Part model, mm, in its own coordinate system. A direction names the side the tool comes from. Coordinates: 2 decimals unless noted, no trailing zeros. Loops run counter-clockwise (first coordinate to the right, second up) from the corner with the lowest first, then second, coordinate; pieces in that order, holes last. Notation, with made-up numbers: (40, 29) -> (96, 29) arc R28 ccw to (96, 50) -> close; hole circle Ø8 at (40, 27). An arc over 180 degrees is marked (long way). One line per item, written item: value. Start each with the question number.
from build123d import *

# Parameters (mm, degrees)
SKETCH_1_R             = 3
EXTRUDE_1_DEPTH        = 71
HOLE_WIZARD_M4_2_D     = 3.3
HOLE_WIZARD_M4_2_DEPTH = 11.5
HOLE_WIZARD_M4_2_TIP   = 0.991420021
CHAMFER_1_SIZE         = 0.5
EXTRUDE1_DEPTH         = 72.126647608
EXTRUDE1_DEPTH_BACK    = 72.126647608
SKETCH1_W              = 2.697137816
SKETCH1_H              = 6
SKETCH1_W_2            = 2.361838602
SKETCH4_R              = 5
SKETCH4_R_2            = 3
EXTRUDE2_DEPTH         = 3


with BuildPart() as part:
    # 草图1 → 凸台-拉伸1 (new body)
    with BuildSketch(Plane.XY):
        Circle(SKETCH_1_R)
    extrude(amount=EXTRUDE_1_DEPTH)

    # M4 螺纹孔2
    with Locations(Plane.XY.offset(71)):
        with Locations((0, 0)):
            Hole(HOLE_WIZARD_M4_2_D / 2, depth=HOLE_WIZARD_M4_2_DEPTH)
            with Locations((0, 0, -(HOLE_WIZARD_M4_2_DEPTH + HOLE_WIZARD_M4_2_TIP / 2))):  # 118° drill point
                Cone(0, HOLE_WIZARD_M4_2_D / 2, HOLE_WIZARD_M4_2_TIP, mode=Mode.SUBTRACT)

    # 倒角1
    chamfer_1_edges = [part.edges().sort_by_distance(p)[0] for p in [
        (-3, 0, 71),
    ]]
    chamfer(chamfer_1_edges, length=CHAMFER_1_SIZE)

    # Sketch1 → Extrude1 (cut, two sides: drawn at the far end of the back side and taken through both)
    with BuildSketch(Plane(origin=(0, 0, 0), x_dir=(1, 0, 0), z_dir=(0, 1, 0)).offset(-EXTRUDE1_DEPTH_BACK)):
        with Locations((-3.848568908, -63)):
            Rectangle(SKETCH1_W, SKETCH1_H)
        with Locations((3.680919301, -63)):
            Rectangle(SKETCH1_W_2, SKETCH1_H)
    extrude(amount=EXTRUDE1_DEPTH + EXTRUDE1_DEPTH_BACK, mode=Mode.SUBTRACT)

    # Sketch4 → Extrude2 (add)
    with BuildSketch(Plane(origin=(0, 0, 0), x_dir=(-1, 0, 0), z_dir=(0, 0, -1))):
        Circle(SKETCH4_R)
        Circle(SKETCH4_R_2, mode=Mode.SUBTRACT)
    extrude(amount=-EXTRUDE2_DEPTH)


solid = part.part
1) Slice it at A-A (x = -4.25). Give the cut face in (y, z).
2) Pin check, flat tips, straight feed: pin 1 Ø3.5 at (y, z) = (-0.5, 62) entering from +X; pin 2 Ø1 at (x, z) = (2.5, 41) entering from +Y; pin 3 Ø3 at (y, z) = (1.5, 13.5) entering from +X. Stop position of each tip, or through.
3) Probe line 1 (Y direction, x = 0, z = 68.5); line 2 (X direction, y = 0, z = 63.75); line 3 (Z direction, x = -2, y = -4). List the from-to ranges inside material, lowest first. Write a range as from..to.
4) Tool access for faces 5 (the cylindrical face through (-3, 0, 36)), 6 (the flat face through (-2.5, 0, 63)), 7 (the flat face through (2, -1, 71)): list every direction of +Z, -Z, +X, -X, +Y, -Y with a clear straight run to the whole face (end or side of a thin tool).
5) Pull direction Y, two halves, no side cores. Call faces 1 (the conical face through (-0.1, -0.3, 58.7)), 2 (the cylindrical face through (1.08, -4.88, 1.48)), 3 (the flat face through (2.5, 0, 63)), 4 (the cylindrical face through (1.216, 1.115, 65.17)): +Y half, -Y half, draft (parallel to the pull), parting line (faces both ways), or undercut.
Check sheet entries:
1. outline: (-2.63, 0) -> (2.63, 0) -> (2.63, 3) -> (-2.63, 3) -> close
2. pin 1: stops at x = 2.5
2. pin 2: stops at y = 2.24
2. pin 3: stops at x = 3
3. line 1: y = -3..-1.65, 1.65..3
3. line 2: x = -2.5..-1.65, 1.65..2.5
3. line 3: z = 0..3
4. face 5: +Z
4. face 6: -X, +Y, -Y
4. face 7: +Z, +X, -X, +Y, -Y
5. face 1: undercut
5. face 2: parting line
5. face 3: draft
5. face 4: undercut
